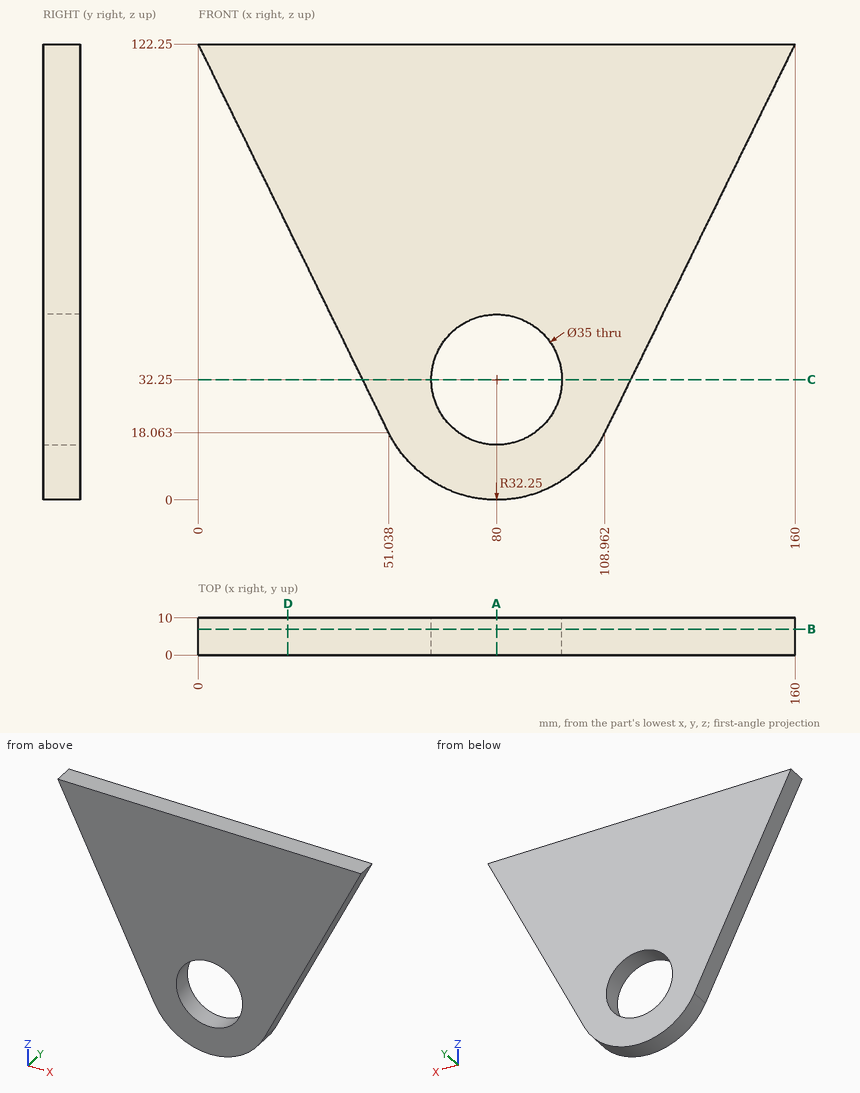
Design review of the part shown in the three views and the two pictorial views. Dimensions are in mm from the part's minimum x, y and z. Round coordinates to 2 decimals unless told otherwise and drop trailing zeros. Order: outer loops, then holes, each group sorted by start corner. A loop starts at its lowest first (then second) coordinate and runs counter-clockwise, first axis right, second up.
Q1. We need section C-C, the plane z = 32.25. Give the boundary of the cut face in (x, y).
Findings below:
outline: (44.09, 0) - (62.5, 0) - (62.5, 10) - (44.09, 10) - close; (97.5, 0) - (115.91, 0) - (115.91, 10) - (97.5, 10) - close
Q2. Wall thickness on line 1 (Z direction, x = 82.5, y = 2); line 2 (X direction, y = 2.5, z = 44); line 3 (X direction, y = 1.25, z = 23.5) (1 decimal): over which ranges is each line inside the solid? List them lowest first.
Findings below:
line 1: z = 0.1 to 14.93, 49.57 to 122.25
line 2: x = 38.33 to 67.03, 92.97 to 121.67
line 3: x = 48.4 to 64.8, 95.2 to 111.6
Q3. We need section B-B, the plane y = 7. Give the boundary of the cut face in (x, z), plus the area to 3 significant figures.
Findings below:
outline: (0, 122.25) - (51.04, 18.06) arc R32.25 ccw to (108.96, 18.06) - (160, 122.25) - close; hole circle Ø35 at (80, 32.25)
area: 11,100 mm2
Q4. We need section A-A, the plane x = 80. Give the boundary of the cut face in (y, z).
Findings below:
outline: (0, 0) - (10, 0) - (10, 14.75) - (0, 14.75) - close; (0, 49.75) - (10, 49.75) - (10, 122.25) - (0, 122.25) - close
Q5. We need section D-D, the plane x = 24. Give the boundary of the cut face in (y, z).
Findings below:
outline: (0, 73.26) - (10, 73.26) - (10, 122.25) - (0, 122.25) - close
Q6. Insertion check: P1, Ø1.5, axis at y = 6.5, z = 79.5, coming from the -X side (1 decimal); P2, Ø3, axis at x = 66.5, y = 2, coming from the -Z side (1 decimal); P3, Ø1.5, axis at y = 3.5, z = 97.5, coming from the -X side. Each pin has a flat end and moves straight along its axis. Give the tip position at first contact, or say it passes through.
Findings below:
P1: stops at x = 20.6
P2: stops at z = 2.3
P3: stops at x = 11.76
